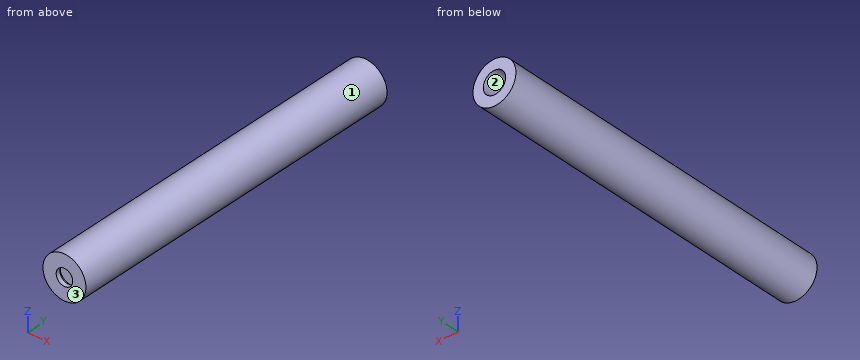
from build123d import *

# Parameters (mm, degrees)
F_25_0_25_DIAMETER_HOLE1_D     = 25
F_25_0_25_DIAMETER_HOLE1_DEPTH = 30
F_25_0_25_DIAMETER_HOLE1_TIP   = 7.510757738


with BuildPart() as part:
    # Sketch1 → Revolve1 (revolve)
    with BuildSketch(Plane(origin=(0, 0, 0), x_dir=(0, 0, -1), z_dir=(1, 0, 0))):
        Polygon((0, 395), (24, 395), (24, 0), (9.25, 0), (9.25, 5), (11.5, 5), (11.5, 8), (0, 8), align=None)
    revolve(axis=Axis((0, 0, 0), (0, 1, 0)))

    # Ø25.0 (25) Diameter Hole1
    with Locations(Plane.ZX.offset(395)):
        with Locations((0, 0)):
            Hole(F_25_0_25_DIAMETER_HOLE1_D / 2, depth=F_25_0_25_DIAMETER_HOLE1_DEPTH)
            with Locations((0, 0, -(F_25_0_25_DIAMETER_HOLE1_DEPTH + F_25_0_25_DIAMETER_HOLE1_TIP / 2))):  # 118° drill point
                Cone(0, F_25_0_25_DIAMETER_HOLE1_D / 2, F_25_0_25_DIAMETER_HOLE1_TIP, mode=Mode.SUBTRACT)


solid = part.part
Geometry check sheet. Reference: the model listing, model coordinates, mm. Face numbers are marked on the shaded views. Round coordinates to 2 decimals unless told otherwise and drop trailing zeros. Write each loop counter-clockwise with the first axis right and the second up, starting at its lowest first coordinate (ties: lowest second). Pieces come first, ordered by that corner, then holes.
Item 1: Material ranges on line 1 along Z through (x, y) = (0, 5.75); line 2 along X through (y, z) = (381, 0); line 3 along Z through (x, y) = (0, 1), recorded low to high.
Determined:
line 1: z = -24 to -11.5, 11.5 to 24
line 2: x = -24 to -12.5, 12.5 to 24
line 3: z = -24 to -9.25, 9.25 to 24
Item 2: Go/stop test with flat-tipped pins: pin 1 Ø6 at (y, z) = (138, 18.5) entering from +X; pin 2 Ø3 at (x, y) = (5, 250.5) entering from -Z; pin 3 Ø16.5 at (x, z) = (0, 0) entering from -Y. Record where each tip stops, or that it passes through.
Determined:
pin 1: stops at x = 18.32
pin 2: stops at z = -23.74
pin 3: stops at y = 8
Item 3: Section check C-C (x = 18.5). Record the boundary of the cut face in (y, z), plus the area to 3 significant figures.
Determined:
outline: (0, -15.29) - (395, -15.29) - (395, 15.29) - (0, 15.29) - close
area: 12,100 mm2
Item 4: Mould release check, pull along Z, two halves, no side actions. Record for the marked faces 1, 2 and 3: +Z half, -Z half, draft (parallel to the pull), parting line (faces both ways), or undercut.
Determined:
face 1: parting line
face 2: undercut
face 3: draft
Item 5: Section check A-A (y = 107.5). Record the boundary of the cut face in (x, z).
Determined:
outline: circle Ø48 at (0, 0)
Item 6: Section check B-B (z = 16). Record the boundary of the cut face in (x, y), plus the area to 3 significant figures.
Determined:
outline: (-17.89, 0) - (17.89, 0) - (17.89, 395) - (-17.89, 395) - close
area: 14,100 mm2
